Drawing for the job (mm, zero at the part's lowest x, y, z). A direction names the side the tool comes from. Give positions to 0.01 mm unless a question says otherwise; leave off trailing zeros. Order: outer loops, then holes, each group sorted by start corner. A loop starts at its lowest first (then second) coordinate and runs counter-clockwise, first axis right, second up. Notation, with made-up numbers: M 26.5,-19.5 L 41.5,-19.5 A20 ccw 41.5,-2.5 Z; hole C 18,14.5 d4. An arc over 180 degrees is marked long. Answer as a JSON object with one key per item and string values.
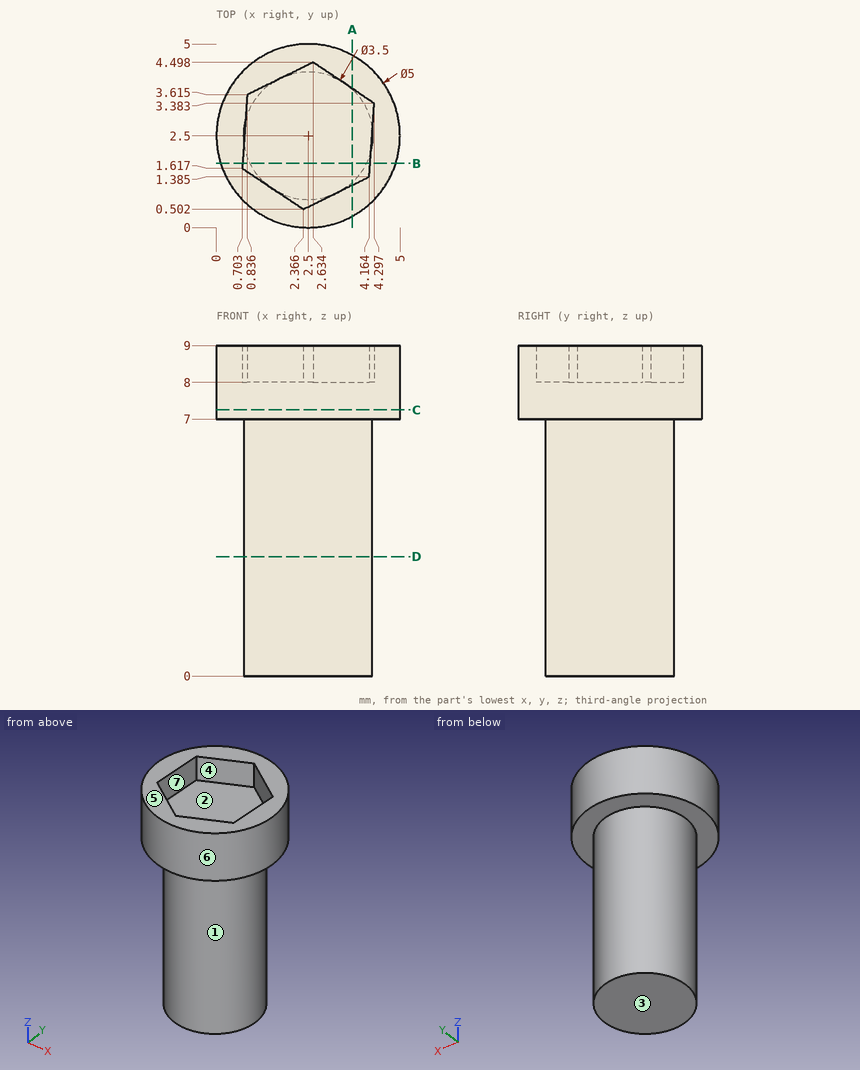
1. Two-plate mould, pull along X, no slides. Class the marked faces 4, 5, 6 and 7: +X half, -X half, draft (parallel to the pull), parting line (faces both ways), or undercut.
Worked answers:
{"face 4": "undercut", "face 5": "draft", "face 6": "parting line", "face 7": "undercut"}
2. Cut at B-B on y = 1.75. Give the cut face in (x, z) (1 decimal), plus the area to 3 significant figures.
Worked answers:
{"outline": "M 0.1,7 L 0.9,7 L 0.9,0 L 4.1,0 L 4.1,7 L 4.9,7 L 4.9,9 L 4.2,9 L 4.2,8 L 0.7,8 L 0.7,9 L 0.1,9 Z", "area": "28.2 mm^2"}
3. Probe line 1 along Y through (x, z) = (2.45, 1.5); line 2 along Z through (x, y) = (3.3, 1.1); line 3 along Z through (x, y) = (1.2, 0.45). List the from-to ranges inside material, lowest first.
Worked answers:
{"line 1": "y = 0.75 to 4.25", "line 2": "z = 0 to 8", "line 3": "z = 7 to 9"}
4. Cut at C-C on z = 7.25. Give the cut face in (x, y), plus the area to 3 significant figures.
Worked answers:
{"outline": "C 2.5,2.5 d5", "area": "19.6 mm^2"}
5. Cut at D-D on z = 3.25. Give the cut face in (x, y).
Worked answers:
{"outline": "C 2.5,2.5 d3.5"}
6. Pin check, flat tips, straight feed: P1, Ø1.5, axis at y = 4.5, z = 4, coming from the +X side (1 decimal); P2, Ø2, axis at x = 1, z = 5, coming from the -Y side. Stop position of each tip, or through.
Worked answers:
{"P1": "stops at x = 3.7", "P2": "stops at y = 0.82"}
7. Cut at A-A on x = 3.7. Give the cut face in (y, z), plus the area to 3 significant figures.
Worked answers:
{"outline": "M 0.31,7 L 1.23,7 L 1.23,0 L 3.77,0 L 3.77,7 L 4.69,7 L 4.69,9 L 3.78,9 L 3.78,8 L 1.16,8 L 1.16,9 L 0.31,9 Z", "area": "24.0 mm^2"}
8. Which spindle directions (+Z, -Z, +X, -X, +Y, -Y) get a long thin tool onto all of the face, cutting with end or side? Do the marked faces 1, 2 and 3. Say none if no direction does.
Worked answers:
{"face 1": "-Z", "face 2": "+Z", "face 3": "-Z, +X, -X, +Y, -Y"}
